Part model, mm, in its own coordinate system. Face numbers are marked on the shaded views. A direction names the side the tool comes from. Give positions to 0.01 mm unless a question says otherwise; leave off trailing zeros. Order: outer loops, then holes, each group sorted by start corner. A loop starts at its lowest first (then second) coordinate and runs counter-clockwise, first axis right, second up. Notation, with made-up numbers: (42, 36) -> (88, 36) arc R22 cw to (88, 51) -> close; hole circle Ø5 at (43.5, 79.25). An arc over 180 degrees is marked (long way). Write item = value, one per line. Start each with the question number.
Item 1: Pull direction X, two halves, no side cores. Call the marked faces 1, 2 and 3: +X half, -X half, draft (parallel to the pull), parting line (faces both ways), or undercut.
Item 2: Band-saw the part on C-C on y = 3.75. Write the cut outline in (x, z), plus the area to 3 significant figures.
Item 3: Band-saw the part on D-D on x = 8. Write the cut outline in (y, z).
Item 4: Drill centre lines: line 1 along Y through (x, z) = (-5, 2); line 2 along Z through (x, y) = (-4, 7.25); line 3 along X through (y, z) = (14.6, 0). Where is each one in solid material? Low to high.
Item 5: Tool access for the marked faces 4, 5, 6 and 7: list every direction of +Z, -Z, +X, -X, +Y, -Y with a clear straight run to the whole face (end or side of a thin tool).
Item 6: Flat gauge pins, fed straight in: P1, Ø8, axis at x = -3, y = 5.5, coming from the -Z side; P2, Ø2.5, axis at x = 8, y = 2.5, coming from the +Z side; P3, Ø3, axis at y = 11.5, z = -4, coming from the +X side; P4, Ø1, axis at x = 3, z = 4.5, coming from the +Y side. Where does each tip first touch, or does it go through?
```python
from build123d import *

# Parameters (mm, degrees)
EXTRUDE_1_DEPTH      = 6
SKETCH_2_R           = 5
EXTRUDE_2_DEPTH      = 4.25
SKETCH_3_R           = 4.625
EXTRUDE_3_DEPTH      = 0.75
SKETCH_4_R           = 5
EXTRUDE_M10_1_DEPTH  = 6.2
SKETCH_5_R           = 4
EXTRUDE_5_DEPTH      = 1.2
SKETCH_6_R           = 3
CUT_EXTRUDE_1_DEPTH  = 5
HOLE_WIZARD_M5_1_D   = 4.2
CHAMFER_C0_25_1_SIZE = 0.25


with BuildPart() as part:
    # 草图1 → 凸台-拉伸1 (new body)
    with BuildSketch(Plane(origin=(0, 0, 0), x_dir=(1, 0, 0), z_dir=(0, 1, 0))):
        with BuildLine():
            Line((6.873863542, 2), (9, 2))
            ThreePointArc((9, 2), (9.707106781, 1.707106781), (10, 1))
            Line((10, 1), (10, -1))
            ThreePointArc((10, -1), (9.707106781, -1.707106781), (9, -2))
            Line((9, -2), (6.873863542, -2))
            ThreePointArc((6.873863542, -2), (6.326140985, -2.163339973), (5.957348403, -2.6))
            ThreePointArc((5.957348403, -2.6), (0, -6.5), (-5.957348403, -2.6))
            ThreePointArc((-5.957348403, -2.6), (-6.326140985, -2.163339973), (-6.873863542, -2))
            Line((-6.873863542, -2), (-9, -2))
            ThreePointArc((-9, -2), (-9.707106781, -1.707106781), (-10, -1))
            Line((-10, -1), (-10, 1))
            ThreePointArc((-10, 1), (-9.707106781, 1.707106781), (-9, 2))
            Line((-9, 2), (-6.873863542, 2))
            ThreePointArc((-6.873863542, 2), (-6.326140985, 2.163339973), (-5.957348403, 2.6))
            ThreePointArc((-5.957348403, 2.6), (0, 6.5), (5.957348403, 2.6))
            ThreePointArc((5.957348403, 2.6), (6.326140985, 2.163339973), (6.873863542, 2))
        make_face()
    extrude(amount=EXTRUDE_1_DEPTH)

    # 草图2 → 凸台-拉伸2 (add)
    with BuildSketch(Plane(origin=(0, 6, 0), x_dir=(1, 0, 0), z_dir=(0, 1, 0))):
        with Locations(Location((0, 0, 0), (0, 0, 270))):
            Circle(SKETCH_2_R)
    extrude(amount=EXTRUDE_2_DEPTH)

    # 草图3 → 凸台-拉伸3 (add)
    with BuildSketch(Plane(origin=(0, 10.25, 0), x_dir=(1, 0, 0), z_dir=(0, 1, 0))):
        with Locations(Location((0, 0, 0), (0, 0, 270))):
            Circle(SKETCH_3_R)
    extrude(amount=EXTRUDE_3_DEPTH)

    # 草图4 → M10×1 细牙螺柱 (add)
    with BuildSketch(Plane(origin=(0, 11, 0), x_dir=(1, 0, 0), z_dir=(0, 1, 0))):
        with Locations(Location((0, 0, 0), (0, 0, 270))):
            Circle(SKETCH_4_R)
    extrude(amount=EXTRUDE_M10_1_DEPTH)

    # 草图5 → 凸台-拉伸5 (add)
    with BuildSketch(Plane(origin=(0, 17.2, 0), x_dir=(1, 0, 0), z_dir=(0, 1, 0))):
        with Locations(Location((0, 0, 0), (0, 0, 270))):
            Circle(SKETCH_5_R)
    extrude(amount=EXTRUDE_5_DEPTH)

    # 草图6 → 切除-拉伸1 (cut)
    with BuildSketch(Plane(origin=(0, 18.4, 0), x_dir=(1, 0, 0), z_dir=(0, 1, 0))):
        with Locations(Location((0, 0, 0), (0, 0, 270))):
            Circle(SKETCH_6_R)
    extrude(amount=-CUT_EXTRUDE_1_DEPTH, mode=Mode.SUBTRACT)

    # M5 螺纹孔1 (through all)
    with Locations(Plane(origin=(0, 0, 0), x_dir=(-1, 0, 0), z_dir=(0, -1, 0))):
        with Locations((0, 0)):
            Hole(HOLE_WIZARD_M5_1_D / 2)

    # C0.25 倒角1
    chamfer_c0_25_1_edges = [part.edges().sort_by_distance(p)[0] for p in [
        (-6.326140985, 6, -2.163339973),
        (-7.936931771, 6, -2),
        (-9.707106781, 6, -1.707106781),
        (-10, 6, 0),
        (-9.707106781, 6, 1.707106781),
        (-7.936931771, 6, 2),
        (-6.326140985, 6, 2.163339973),
        (0, 6, 6.5),
        (6.326140985, 6, 2.163339973),
        (0, 10.25, -5),
        (7.936931771, 6, 2),
        (6.326140985, 6, -2.163339973),
        (9.707106781, 6, 1.707106781),
        (10, 6, 0),
        (9.707106781, 6, -1.707106781),
        (7.936931771, 6, -2),
        (0, 18.4, -3),
        (0, 6, -6.5),
    ]]
    chamfer(chamfer_c0_25_1_edges, length=CHAMFER_C0_25_1_SIZE)


solid = part.part
```
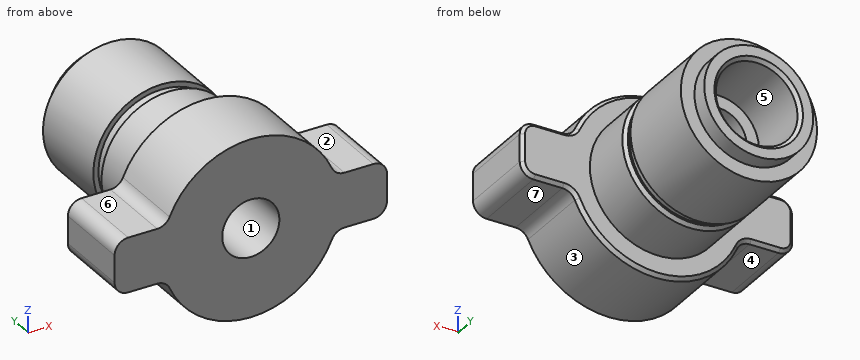
Values found:
q1.face_1 = undercut
q1.face_2 = draft
q1.face_3 = parting line
q2.outline = (-10, -1) arc R1 ccw to (-9, -2) -> (-6.87, -2) arc R1 cw to (-5.96, -2.6) arc R6.5 ccw to (5.96, -2.6) arc R1 cw to (6.87, -2) -> (9, -2) arc R1 ccw to (10, -1) -> (10, 1) arc R1 ccw to (9, 2) -> (6.87, 2) arc R1 cw to (5.96, 2.6) arc R6.5 ccw to (-5.96, 2.6) arc R1 cw to (-6.87, 2) -> (-9, 2) arc R1 ccw to (-10, 1) -> close; hole circle Ø4.2 at (0, 0)
q2.area = 147 mm^2
q3.outline = (0, -2) -> (5.75, -2) -> (6, -1.75) -> (6, 1.75) -> (5.75, 2) -> (0, 2) -> close
q4.line_1 = 0 to 6
q4.line_2 = -3 to 3
q4.line_3 = -5 to -3, 3 to 5
q5.face_4 = -Z, -X, +Y, -Y
q5.face_5 = +Y
q5.face_6 = +Z, -X, +Y, -Y
q5.face_7 = -Z, +X, +Y, -Y
q6.P1 = -6.5
q6.P2 = 2.01
q6.P3 = 4.33
q6.P4 = 17.2
